Verification items for the finished model (mm, model axes). Face numbers are marked on the shaded views. Coordinates: 2 decimals unless noted, no trailing zeros. Write each loop counter-clockwise with the first axis right and the second up, starting at its lowest first coordinate (ties: lowest second). Pieces come first, ordered by that corner, then holes. Notation, with made-up numbers: M -19,4 L 19,4 A16 cw 19,22 Z; hole C 52,70.25 d9. An arc over 180 degrees is marked long. Answer in a Markdown table with one row per item.
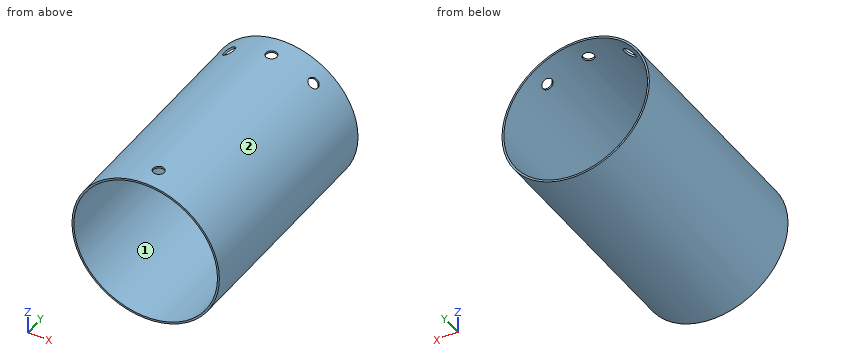
from build123d import *

# Parameters (mm, degrees)
SKETCH_2_R          = 79.5
SKETCH_2_R_2        = 77.5
EXTRUDE_1_DEPTH     = 123
SKETCH_3_R          = 6
CUT_EXTRUDE_2_DEPTH = 167.641831483
SKETCH_4_R          = 6
CUT_EXTRUDE_3_DEPTH = 167.641831653
SKETCH_5_R          = 7
CUT_EXTRUDE_4_DEPTH = 167.641831653


with BuildPart() as part:
    # 草图2 → 拉伸-薄壁1 (new, symmetric)
    with BuildSketch(Plane(origin=(0, 0, 0), x_dir=(1, 0, 0), z_dir=(0, 1, 0))):
        Circle(SKETCH_2_R)
        Circle(SKETCH_2_R_2, mode=Mode.SUBTRACT)
    extrude(amount=EXTRUDE_1_DEPTH, both=True)

    # 草图3 → 切除-拉伸2 (cut, through all)
    with BuildSketch(Plane.XY):
        with Locations(Location((0, 100, 0), (0, 0, 180))):
            Circle(SKETCH_3_R)
        with Locations(Location((0, -100, 0), (0, 0, 180))):
            Circle(SKETCH_3_R)
    extrude(amount=CUT_EXTRUDE_2_DEPTH, mode=Mode.SUBTRACT)

    # 草图4 → 切除-拉伸3 (cut, through all)
    with BuildSketch(Plane(origin=(0, 0, 0), x_dir=(0, -1, 0), z_dir=(0.5735764363510444, 0, 0.819152044288993))):
        with Locations(Location((-100, 0, 0), (0, 0, 270))):
            Circle(SKETCH_4_R)
    extrude(amount=CUT_EXTRUDE_3_DEPTH, mode=Mode.SUBTRACT)

    # 草图5 → 切除-拉伸4 (cut, through all)
    with BuildSketch(Plane(origin=(0, 0, 0), x_dir=(0, -1, 0), z_dir=(0.5735764363510444, 0, -0.819152044288993))):
        with Locations(Location((-100, 0, 0), (0, 0, 90))):
            Circle(SKETCH_5_R)
    extrude(amount=-CUT_EXTRUDE_4_DEPTH, mode=Mode.SUBTRACT)


solid = part.part
1) Depth check by flat-ended pin: pin 1 (2 mm diameter, centred on x = -59.5, y = 51.5, fed in from -Z); pin 2 (5 mm diameter, centred on x = 20.5, y = 6, fed in from -Z); pin 3 (1.5 mm diameter, centred on y = -24, z = 3.5, fed in from -X). Enter the tip coordinate at first touch or a pass-through.
Response values:
| item | result |
|---|---|
| pin 1 | stops at z = -53.83 |
| pin 2 | stops at z = -77.44 |
| pin 3 | stops at x = -79.45 |
2) Thickness scan on L1, parallel to Y at x = 0, z = 78; L2, parallel to X at y = 70, z = 0. Record the ranges inside material, lowest first. Write a range as [from, to].
Response values:
| item | result |
|---|---|
| L1 | y = [-123, -106], [-94, 94], [106, 123] |
| L2 | x = [-79.5, -77.5], [77.5, 79.5] |
3) Sectioned sample at D-D (y = 100). Record the cut outline in (x, z), then the cut area to 3 significant figures.
Response values:
| item | result |
|---|---|
| outline | M -51.16,60.85 A79.5 ccw long 50.38,61.5 L 49.23,59.85 A77.5 cw long -50,59.21 Z; M -39.69,68.88 L -38.54,67.24 A77.5 cw -6,77.27 L -6,79.27 A79.5 ccw Z; M 6,77.27 A77.5 cw 39.4,66.74 L 40.55,68.38 A79.5 ccw 6,79.27 Z |
| area | 910 mm² |
4) Release check for a two-part mould opening along X. For the marked faces 1 and 2 record: +X half, -X half, draft (parallel to the pull), parting line (faces both ways), or undercut.
Response values:
| item | result |
|---|---|
| face 1 | undercut |
| face 2 | parting line |
5) Sectioned sample at A-A (z = 0). Record the cut outline in (x, y), then the cut area to 3 significant figures.
Response values:
| item | result |
|---|---|
| outline | M -79.5,-123 L -77.5,-123 L -77.5,123 L -79.5,123 Z; M 77.5,-123 L 79.5,-123 L 79.5,123 L 77.5,123 Z |
| area | 984 mm² |
6) Sectioned sample at C-C (x = 67). Record the cut outline in (y, z), then the cut area to 3 significant figures.
Response values:
| item | result |
|---|---|
| outline | M -123,-42.79 L 123,-42.79 L 123,-38.95 L -123,-38.95 Z; M -123,38.95 L 123,38.95 L 123,42.79 L -123,42.79 Z |
| area | 1,890 mm² |
7) Sectioned sample at B-B (x = 0). Record the cut outline in (y, z).
Response values:
| item | result |
|---|---|
| outline | M -123,-79.5 L 123,-79.5 L 123,-77.5 L -123,-77.5 Z; M -123,77.5 L -106,77.5 L -106,79.5 L -123,79.5 Z; M -94,77.5 L 94,77.5 L 94,79.5 L -94,79.5 Z; M 106,77.5 L 123,77.5 L 123,79.5 L 106,79.5 Z |
